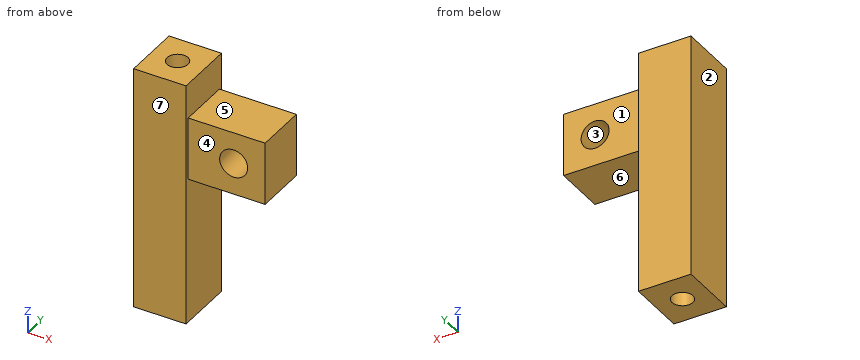
```python
from build123d import *

# Parameters (mm, degrees)
SKETCH1_W           = 22
SKETCH1_H           = 15
BOSS_EXTRUDE1_DEPTH = 18
SKETCH2_W           = 70
SKETCH2_H           = 17
BOSS_EXTRUDE2_DEPTH = 15
SKETCH4_R           = 3
CUT_EXTRUDE2_DEPTH  = 110
SKETCH3_R           = 4
CUT_EXTRUDE4_DEPTH  = 41


with BuildPart() as part:
    # Sketch1 → Boss-Extrude1 (new body)
    with BuildSketch(Plane.XY):
        with Locations((-13, -1.305964762)):
            Rectangle(SKETCH1_W, SKETCH1_H)
    extrude(amount=BOSS_EXTRUDE1_DEPTH)

    # Sketch2 → Boss-Extrude2 (add)
    with BuildSketch(Plane.ZY.offset(24)):
        with Locations((-7, -1.305964762)):
            Rectangle(SKETCH2_W, SKETCH2_H)
    extrude(amount=BOSS_EXTRUDE2_DEPTH)

    # Sketch4 → Cut-Extrude2 (cut)
    with BuildSketch(Plane.XY.offset(28)):
        with Locations((-31.5, -1.305964762)):
            Circle(SKETCH4_R)
    extrude(amount=-CUT_EXTRUDE2_DEPTH, mode=Mode.SUBTRACT)

    # Sketch3 → Cut-Extrude4 (cut)
    with BuildSketch(Plane(origin=(0, 6.194035238, 0), x_dir=(1, 0, 0), z_dir=(0, 1, 0))):
        with Locations(Location((-11, -9, 0), (0, 0, 270))):
            Circle(SKETCH3_R)
    extrude(amount=-CUT_EXTRUDE4_DEPTH, mode=Mode.SUBTRACT)


solid = part.part
```
Geometry: final body of the model. Coordinates: model frame, mm. Face numbers are marked on the shaded views. A direction names the side the tool comes from. Coordinates: 2 decimals unless noted, no trailing zeros. Order: outer loops, then holes, each group sorted by start corner. A loop starts at its lowest first (then second) coordinate and runs counter-clockwise, first axis right, second up. Notation, with made-up numbers: (-14, -27.75) -> (-3, -27.75) arc R34 ccw to (-3, 9.25) -> close; hole circle Ø9 at (79, 67.25). An arc over 180 degrees is marked (long way). Write each question's results on one line, items separated by ' | '. Start each with the question number.
1) Cut plane C-C, the plane y = -0.25. Output: boundary loops of the cut face in (x, z).
2) Cut plane D-D, the plane z = 9. Output: boundary loops of the cut face in (x, y), and give its area (3 significant figures).
3) Cut plane A-A, the plane x = -31.5. Output: boundary loops of the cut face in (y, z), and give its area (3 significant figures).
4) First-contact query: pin 1 (1.5 mm diameter, centred on y = 2, z = -34.5, fed in from +X); pin 2 (1.5 mm diameter, centred on x = -15, y = 0.5, fed in from -Z); pin 3 (5.5 mm diameter, centred on x = -14, z = 5, fed in from -Y); pin 4 (6 mm diameter, centred on y = -7.5, z = -1, fed in from +X). Flat tips, straight axial feed; report the tip coordinate or a pass-through.
5) Cut plane B-B, the plane y = 3. Output: boundary loops of the cut face in (x, z).
6) Set-up query: the marked faces 4, 5, 6 and 7. Return all of +Z, -Z, +X, -X, +Y, -Y with unobstructed straight access to the full face (end or side cutting, diameter ignored); none if empty.
7) Material intervals for line 1 along X through (y, z) = (-1.5, 9); line 2 along X through (y, z) = (3.25, 9); line 3 along X through (y, z) = (-3, 8.5), sorted ascending.
8) Mould query, pull axis X, two halves, no side actions, for the marked faces 1, 2 and 3. Classes: released by +X, released by -X, zero draft, split by the parting line, or undercut.
Checks:
1) outline: (-39, -42) -> (-34.31, -42) -> (-34.31, 28) -> (-39, 28) -> close; (-28.69, -42) -> (-24, -42) -> (-24, 0) -> (-2, 0) -> (-2, 18) -> (-24, 18) -> (-24, 28) -> (-28.69, 28) -> close; hole circle Ø8 at (-11, 9)
2) outline: (-39, -9.81) -> (-24, -9.81) -> (-24, -8.81) -> (-15, -8.81) -> (-15, 6.19) -> (-24, 6.19) -> (-24, 7.19) -> (-39, 7.19) -> close; (-7, -8.81) -> (-2, -8.81) -> (-2, 6.19) -> (-7, 6.19) -> close; hole circle Ø6 at (-31.5, -1.31) | area: 437 mm^2
3) outline: (-9.81, -42) -> (-4.31, -42) -> (-4.31, 28) -> (-9.81, 28) -> close; (1.69, -42) -> (7.19, -42) -> (7.19, 28) -> (1.69, 28) -> close | area: 770 mm^2
4) pin 1: x = -24 | pin 2: z = 0 | pin 3: y = -8.81 | pin 4: x = -2
5) outline: (-39, -42) -> (-24, -42) -> (-24, 0) -> (-2, 0) -> (-2, 18) -> (-24, 18) -> (-24, 28) -> (-39, 28) -> close; hole circle Ø8 at (-11, 9)
6) face 4: +Z, -Z, +X, -Y | face 5: +Z, +X, +Y, -Y | face 6: -Z, +X, +Y, -Y | face 7: +Z, -Z, +X, -X, -Y
7) line 1: -39 to -34.49, -28.51 to -15, -7 to -2 | line 2: -39 to -15, -7 to -2 | line 3: -39 to -33.98, -29.02 to -14.97, -7.03 to -2
8) face 1: zero draft | face 2: released by -X | face 3: undercut
